Part print with two shaded views. Sizes in mm from the minimum x, y, z corner. A direction names the side the tool comes from. Round coordinates to 2 decimals unless told otherwise and drop trailing zeros. Order: outer loops, then holes, each group sorted by start corner. A loop starts at its lowest first (then second) coordinate and runs counter-clockwise, first axis right, second up. Notation, with made-up numbers: (25, -17.75) - (33, -17.75) arc R27 cw to (33, 4.25) - close; hole circle Ø9 at (61, 28.5). An arc over 180 degrees is marked (long way). Write item = value, one per line.
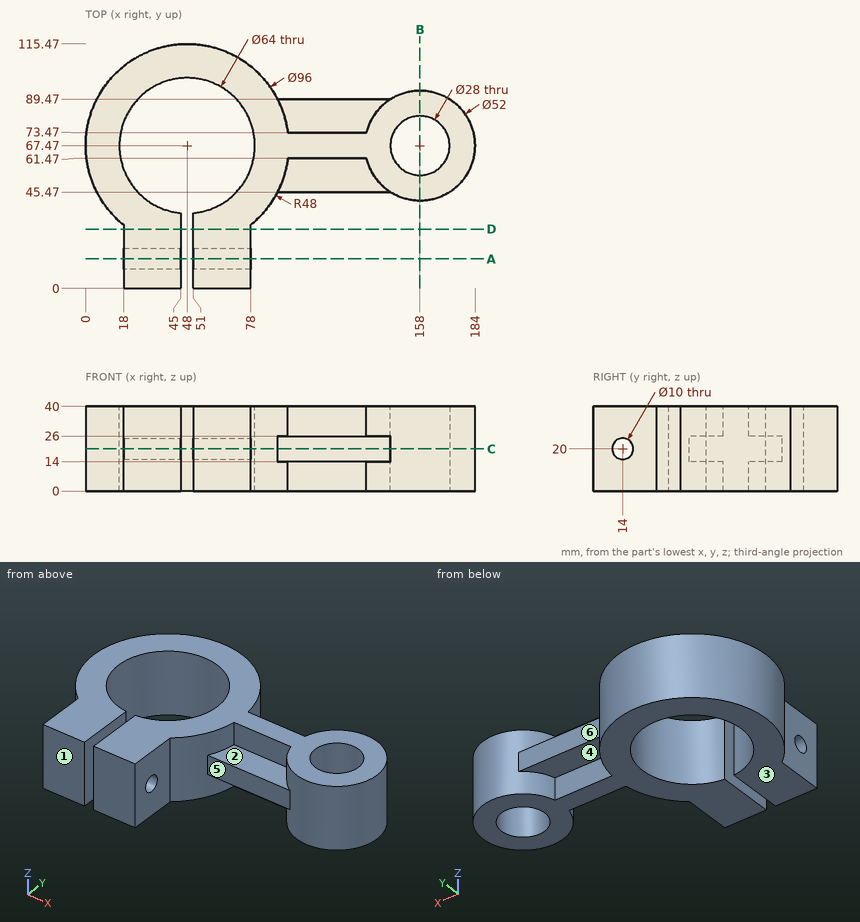
1) Wall check: line 1 along X through (y, z) = (67, 9); line 2 along Z through (x, y) = (57.25, 14); line 3 along X through (y, z) = (16, 4.5). Give the ranges that are in metal, low to high.
Conclusion:
line_1 = 0 to 16, 80 to 144.01, 171.99 to 184
line_2 = 0 to 15, 25 to 40
line_3 = 18 to 45, 51 to 78
2) 3-axis set-ups, long thin cutter, end or side, ignore diameter. For the marked faces 4, 5 and 6: which of +Z, -Z, +X, -X, +Y, -Y reach the whole face in a straight line?
Conclusion:
face_4 = -Z, +Y
face_5 = +Z, -Z, -Y
face_6 = +Z, -Z, +Y
3) Flat gauge pins, fed straight in: pin 1 Ø12 at (x, z) = (45.5, 5.5) entering from +Y; pin 2 Ø13 at (x, y) = (109.5, 51.5) entering from +Z; pin 3 Ø8 at (y, z) = (14, 20) entering from +X; pin 4 Ø4 at (x, z) = (117, 5.5) entering from -Y. Where does each tip first touch, or does it go through?
Conclusion:
pin_1 = 115.47
pin_2 = 26
pin_3 = through
pin_4 = 61.47
4) Cut at C-C (z = 20). Write the cut outline in (x, y).
Conclusion:
outline = (18, 0) - (45, 0) - (45, 9) - (18, 9) - close; (18, 19) - (45, 19) - (45, 35.61) arc R32 cw (long way) to (51, 35.61) - (51, 19) - (78, 19) - (78, 30) arc R48 ccw to (90.66, 45.47) - (144.14, 45.47) arc R26 ccw (long way) to (144.14, 89.47) - (90.66, 89.47) arc R48 ccw (long way) to (18, 30) - close; (51, 0) - (78, 0) - (78, 9) - (51, 9) - close; hole circle Ø28 at (158, 67.47)
5) Cut at A-A (y = 14). Write the cut outline in (x, z), and give its area (3 significant figures).
Conclusion:
outline = (18, 0) - (45, 0) - (45, 15) - (18, 15) - close; (18, 25) - (45, 25) - (45, 40) - (18, 40) - close; (51, 0) - (78, 0) - (78, 15) - (51, 15) - close; (51, 25) - (78, 25) - (78, 40) - (51, 40) - close
area = 1,620 mm^2
6) Mould opens along Z. For the marked faces 1, 2 and 3 say: +Z half, -Z half, draft (parallel to the pull), parting line (faces both ways), or undercut.
Conclusion:
face_1 = draft
face_2 = +Z half
face_3 = -Z half
7) Cut at D-D (y = 28). Write the cut outline in (x, z).
Conclusion:
outline = (18, 0) - (45, 0) - (45, 40) - (18, 40) - close; (51, 0) - (78, 0) - (78, 40) - (51, 40) - close
8) Cut at B-B (x = 158). Write the cut outline in (y, z), and give its area (3 significant figures).
Conclusion:
outline = (41.47, 0) - (53.47, 0) - (53.47, 40) - (41.47, 40) - close; (81.47, 0) - (93.47, 0) - (93.47, 40) - (81.47, 40) - close
area = 960 mm^2
